The figure shows three views and two pictorial views of one solid part (mm, origin at its lowest corner). Answer the questions. Coordinates: 2 decimals unless noted, no trailing zeros. Loops run counter-clockwise (first coordinate to the right, second up) from the corner with the lowest first, then second, coordinate; pieces in that order, holes last. Notation, with made-up numbers: M -10,43 L -6,43 A35 ccw -6,80 Z; hole C -6,71 d8. An arc over 180 degrees is marked long. Answer as a JSON object with one key per item and string values. Group by question number.
1. Straight lines are drawn through the part: L1, parallel to Y at x = 25, z = 1.45; L2, parallel to Y at x = 25, z = 2.1; L3, parallel to Y at x = 45, z = 1.25. For each, find the intervals that lie inside material, in ascending order.
2. A cutting plane is placed at B-B on z = 2.5. Give the vertices of the cut face in (x, y), and give its area (3 significant figures).
3. Determine the mould class of the marked faces 1, 2 and 3 for opening direction Y: released by +Y, released by -Y, zero draft, split by the parting line, or undercut.
4. A cutting plane is placed at C-C on y = 23.5. State how many separate pieces and enclosed holes the cut face has, and give its area (3 significant figures).
5. A cutting plane is placed at A-A on x = 25. Give the vertices of the cut face in (y, z), and give its area (3 significant figures).
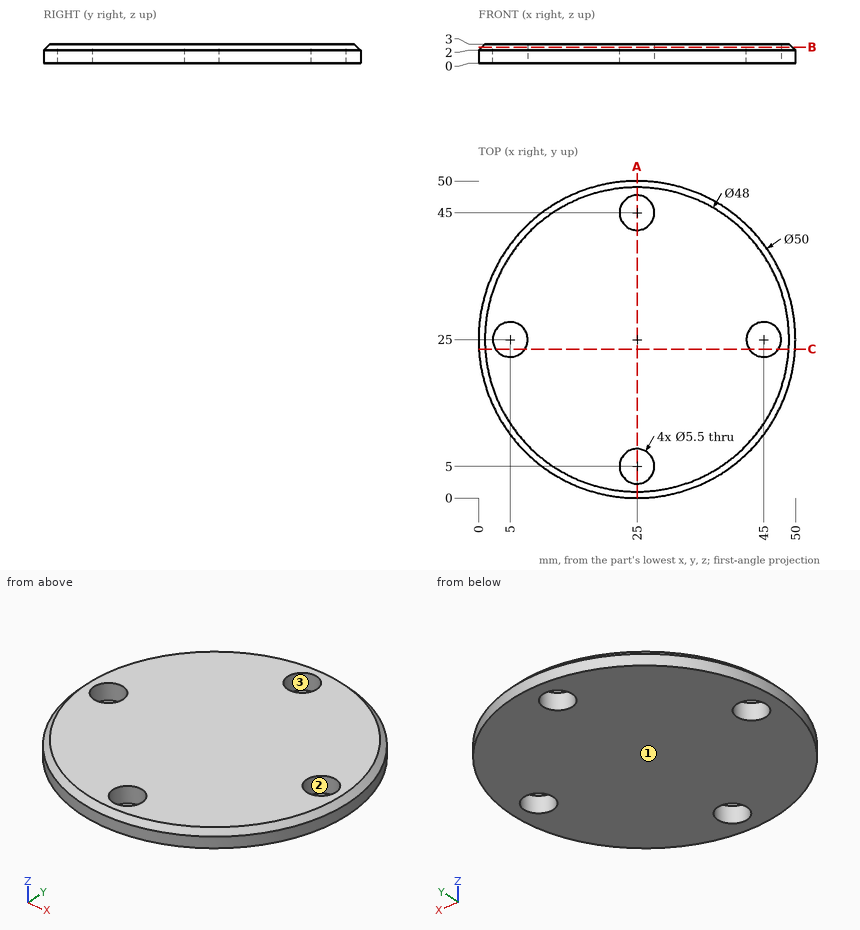
From the geometry:
{
 "1": {"L1": "y = 0 to 2.25, 7.75 to 42.25, 47.75 to 50", "L2": "y = 0.1 to 2.25, 7.75 to 42.25, 47.75 to 49.9", "L3": "y = 10 to 22.25, 27.75 to 40"},
 "2": {"outline": "C 25,25 d49; hole C 5,25 d5.5; hole C 25,5 d5.5; hole C 25,45 d5.5; hole C 45,25 d5.5", "area": "1,790 mm²"},
 "3": {"face 1": "zero draft", "face 2": "undercut", "face 3": "undercut"},
 "4": {"separate pieces": "3", "enclosed holes": "0", "area": "121 mm²"},
 "5": {"outline": "M 0,0 L 2.25,0 L 2.25,3 L 1,3 L 0,2 Z; M 7.75,0 L 42.25,0 L 42.25,3 L 7.75,3 Z; M 47.75,0 L 50,0 L 50,2 L 49,3 L 47.75,3 Z", "area": "116 mm²"}
}
